Drawing for the job (mm, zero at the part's lowest x, y, z). A direction names the side the tool comes from. Coordinates: 2 decimals unless noted, no trailing zeros. Loops run counter-clockwise (first coordinate to the right, second up) from the corner with the lowest first, then second, coordinate; pieces in that order, holes last. Notation, with made-up numbers: (-0.5, 12) - (27.5, 12) arc R24 cw to (27.5, 29) - close; hole circle Ø7 at (79, 50.25). An arc over 180 degrees is marked (long way). One line per item, written item: value.
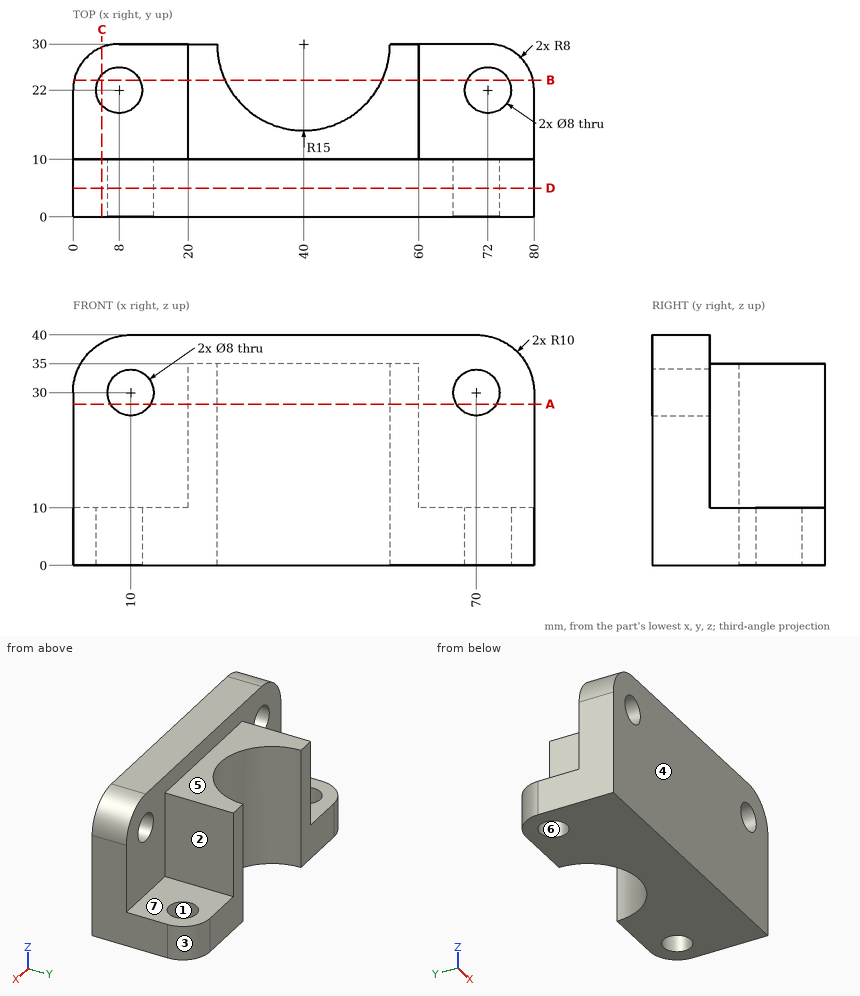
Item 1: Cut at C-C, the plane x = 5. Write the cut outline in (y, z), then the cut area to 3 significant figures.
Check result:
outline: (0, 0) - (19.35, 0) - (19.35, 10) - (10, 10) - (10, 38.66) - (0, 38.66) - close; (24.65, 0) - (29.42, 0) - (29.42, 10) - (24.65, 10) - close
area: 528 mm^2
Item 2: Cut at A-A, the plane z = 28. Write the cut outline in (x, y).
Check result:
outline: (0, 0) - (6.54, 0) - (6.54, 10) - (0, 10) - close; (13.46, 0) - (66.54, 0) - (66.54, 10) - (60, 10) - (60, 30) - (55, 30) arc R15 cw to (25, 30) - (20, 30) - (20, 10) - (13.46, 10) - close; (73.46, 0) - (80, 0) - (80, 10) - (73.46, 10) - close
Item 3: Pull direction Y, two halves, no side cores. Call the marked faces 1, 2, 3 and 4: released by +Y, released by -Y, zero draft, split by the parting line, or undercut.
Check result:
face 1: undercut
face 2: zero draft
face 3: released by +Y
face 4: released by -Y
Item 4: Drop flat-ended pins along their axis: P1, Ø6, axis at x = 7.5, y = 16, coming from the +Z side; P2, Ø16, axis at y = 20.5, z = 28, coming from the +X side; P3, Ø1, axis at x = 30, y = 13.5, coming from the +Z side. Give the stop position or say it passes through.
Check result:
P1: stops at z = 10
P2: stops at x = 60
P3: stops at z = 35
Item 5: Cut at B-B, the plane y = 23.75. Write the cut outline in (x, z), then the cut area to 3 significant figures.
Check result:
outline: (0.19, 0) - (4.4, 0) - (4.4, 10) - (0.19, 10) - close; (11.6, 0) - (26.36, 0) - (26.36, 35) - (20, 35) - (20, 10) - (11.6, 10) - close; (53.64, 0) - (68.4, 0) - (68.4, 10) - (60, 10) - (60, 35) - (53.64, 35) - close; (75.6, 0) - (79.81, 0) - (79.81, 10) - (75.6, 10) - close
area: 698 mm^2
Item 6: Tool access for the marked faces 5, 6 and 7: list every direction of +Z, -Z, +X, -X, +Y, -Y with a clear straight run to the whole face (end or side of a thin tool).
Check result:
face 5: +Z, +X, -X, +Y
face 6: +Z, -Z
face 7: +Z, +X, +Y
Item 7: Probe probe 1 along X at (y, z) = (7.75, 30); probe 2 along Y at (x, z) = (8, 2.75); probe 3 along Z at (x, y) = (59, 13). List the from-to ranges inside material, lowest first. Write a range as from..to.
Check result:
probe 1: x = 0..6, 14..66, 74..80
probe 2: y = 0..18, 26..30
probe 3: z = 0..35
Item 8: Cut at D-D, the plane y = 5. Write the cut outline in (x, z), then the cut area to 3 significant figures.
Check result:
outline: (0, 0) - (80, 0) - (80, 30) arc R10 ccw to (70, 40) - (10, 40) arc R10 ccw to (0, 30) - close; hole circle Ø8 at (10, 30); hole circle Ø8 at (70, 30)
area: 3,060 mm^2
